Check sheet for the modelled part. Datum: model origin and axes. Units: mm. Coordinates: 2 decimals unless noted, no trailing zeros. Order: outer loops, then holes, each group sorted by start corner. A loop starts at its lowest first (then second) coordinate and runs counter-clockwise, first axis right, second up.
1. Cross-section at C-C (z = 4). Enter the section's corners in (x, y).
2. Cross-section at B-B (x = 45). Enter the section's corners in (y, z), then the cut area to 3 significant figures.
3. Cross-section at A-A (y = 0). Enter the section's corners in (x, z), then the cut area to 3 significant figures.
4. Thickness scan on line 1 (Y direction, x = -45, z = 4.75); line 2 (X direction, y = 100.5, z = 4); line 3 (Y direction, x = -48, z = 5.5). Record the ranges inside material, lowest first.
```python
from build123d import *

# Parameters (mm, degrees)
SKETCH1_W           = 150
SKETCH1_H           = 300
SKETCH1_R           = 8
BOSS_EXTRUDE1_DEPTH = 10


with BuildPart() as part:
    # Sketch1 → Boss-Extrude1 (new body)
    with BuildSketch(Plane.XY):
        Rectangle(SKETCH1_W, SKETCH1_H)
        with Locations((-45, 100)):
            Circle(SKETCH1_R, mode=Mode.SUBTRACT)
        with Locations((-45, 0)):
            Circle(SKETCH1_R, mode=Mode.SUBTRACT)
        with Locations((-45, -100)):
            Circle(SKETCH1_R, mode=Mode.SUBTRACT)
        with Locations(Location((45, -100, 0), (0, 0, 180))):
            Circle(SKETCH1_R, mode=Mode.SUBTRACT)
        with Locations(Location((45, 0, 0), (0, 0, 180))):
            Circle(SKETCH1_R, mode=Mode.SUBTRACT)
        with Locations(Location((45, 100, 0), (0, 0, 180))):
            Circle(SKETCH1_R, mode=Mode.SUBTRACT)
    extrude(amount=BOSS_EXTRUDE1_DEPTH)


solid = part.part
```
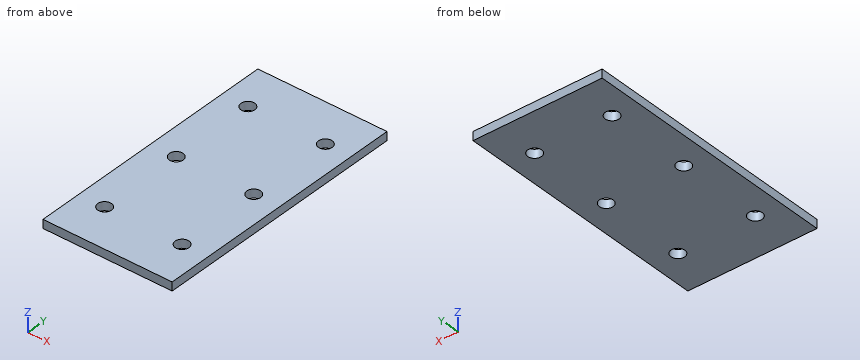
Data:
1. outline: (-75, -150) - (75, -150) - (75, 150) - (-75, 150) - close; hole circle Ø16 at (-45, -100); hole circle Ø16 at (-45, 0); hole circle Ø16 at (-45, 100); hole circle Ø16 at (45, -100); hole circle Ø16 at (45, 0); hole circle Ø16 at (45, 100)
2. outline: (-150, 0) - (-108, 0) - (-108, 10) - (-150, 10) - close; (-92, 0) - (-8, 0) - (-8, 10) - (-92, 10) - close; (8, 0) - (92, 0) - (92, 10) - (8, 10) - close; (108, 0) - (150, 0) - (150, 10) - (108, 10) - close
2. area: 2,520 mm2
3. outline: (-75, 0) - (-53, 0) - (-53, 10) - (-75, 10) - close; (-37, 0) - (37, 0) - (37, 10) - (-37, 10) - close; (53, 0) - (75, 0) - (75, 10) - (53, 10) - close
3. area: 1,180 mm2
4. line 1: y = -150 to -108, -92 to -8, 8 to 92, 108 to 150
4. line 2: x = -75 to -52.98, -37.02 to 37.02, 52.98 to 75
4. line 3: y = -150 to -107.42, -92.58 to -7.42, 7.42 to 92.58, 107.42 to 150
